Verification items for the finished model (mm, model axes). Give positions to 0.01 mm unless a question says otherwise; leave off trailing zeros. Loops run counter-clockwise (first coordinate to the right, second up) from the corner with the lowest first, then second, coordinate; pieces in that order, holes last. Notation, with made-up numbers: (-37.5, 44) -> (1.5, 44) arc R38 cw to (1.5, 82) -> close; hole circle Ø9 at (73.25, -10.75). An arc over 180 degrees is marked (long way). Answer in a Markdown table with one row per item. Add a question column.
Q1. Gauge pin test, flat ends, axial feed: P1, Ø1, axis at y = 1.5, z = 1.5, coming from the -X side; P2, Ø8, axis at x = 7, y = -4.5, coming from the -Z side; P3, Ø1.5, axis at x = 1, y = -4.5, coming from the -Z side. Record the tip position at first contact, or that the pin passes through.
Q2. Section check D-D on x = -6.5. Enter the section's corners in (y, z).
Q3. Material ranges on probe 1 along Y at (x, z) = (0, 2.5); probe 2 along X at (y, z) = (1.25, 7.25); probe 3 along Y at (x, z) = (-2.5, 4), recorded low to high.
Q4. Section check A-A on x = 0. Enter the section's corners in (y, z).
Q5. Section check B-B on y = 5.25. Enter the section's corners in (x, z).
Q6. Section check C-C on z = 1.75. Enter the section's corners in (x, y).
Q7. Release check for a two-part mould opening along Y. For faces 1 (the face through (1.9, 5.4, 8.5)), 2 (the face through (-1.19, -5.37, 4.31)), 3 (the face through (6.961, 3.944, 4.19)), 4 (the face through (6.896, -4.056, 4.19)) record: pulls with the +Y half, pulls with the -Y half, needs draft (parallel to the pull), parting line crosses it, or undercut.
```python
from build123d import *

# Parameters (mm, degrees)
EXTRUDE_1_DEPTH     = 8.5
SKETCH_2_R          = 5.5
CUT_EXTRUDE_1_DEPTH = 8.5


with BuildPart() as part:
    # 草图1 → 凸台-拉伸1 (new body)
    with BuildSketch(Plane.XY):
        Polygon((9.237604307, 0), (4.618802154, 8), (-4.618802154, 8), (-9.237604307, 0), (-4.618802154, -8), (4.618802154, -8), align=None)
    extrude(amount=EXTRUDE_1_DEPTH)

    # 草图2 → 切除-拉伸1 (cut)
    with BuildSketch(Plane.XY.offset(8.5)):
        Circle(SKETCH_2_R)
    extrude(amount=-CUT_EXTRUDE_1_DEPTH, mode=Mode.SUBTRACT)


solid = part.part
```
Taken from the geometry:
| question | item | result |
|---|---|---|
| 1 | P1 | stops at x = -8.66 |
| 1 | P2 | stops at z = 0 |
| 1 | P3 | passes through |
| 2 | outline | (-4.74, 0) -> (4.74, 0) -> (4.74, 8.5) -> (-4.74, 8.5) -> close |
| 3 | probe 1 | y = -8 to -5.5, 5.5 to 8 |
| 3 | probe 2 | x = -8.52 to -5.36, 5.36 to 8.52 |
| 3 | probe 3 | y = -8 to -4.9, 4.9 to 8 |
| 4 | outline | (-8, 0) -> (-5.5, 0) -> (-5.5, 8.5) -> (-8, 8.5) -> close; (5.5, 0) -> (8, 0) -> (8, 8.5) -> (5.5, 8.5) -> close |
| 5 | outline | (-6.21, 0) -> (-1.64, 0) -> (-1.64, 8.5) -> (-6.21, 8.5) -> close; (1.64, 0) -> (6.21, 0) -> (6.21, 8.5) -> (1.64, 8.5) -> close |
| 6 | outline | (-9.24, 0) -> (-4.62, -8) -> (4.62, -8) -> (9.24, 0) -> (4.62, 8) -> (-4.62, 8) -> close; hole circle Ø11 at (0, 0) |
| 7 | face 1 | needs draft |
| 7 | face 2 | undercut |
| 7 | face 3 | pulls with the +Y half |
| 7 | face 4 | pulls with the -Y half |
